Build history of the part. All positions in model axes, mm. A direction names the side the tool comes from. Round coordinates to 2 decimals unless told otherwise and drop trailing zeros. Loops run counter-clockwise (first coordinate to the right, second up) from the corner with the lowest first, then second, coordinate; pieces in that order, holes last. Notation, with made-up numbers: (82.5, 18.5) -> (87.5, 18.5) arc R20 cw to (87.5, 37.5) -> close; hole circle Ø4 at (27.25, -33.5). An arc over 180 degrees is marked (long way). Put each result on its own line as item: value. Start each with the question number.
```python
from build123d import *

# Parameters (mm, degrees)
SKETCH_1_W          = 480
SKETCH_1_H          = 178
EXTRUDE_1_DEPTH     = 2
SKETCH_2_R          = 3
CUT_EXTRUDE_1_DEPTH = 256.978514723
FILLET_1_R          = 5
SKETCH_3_W          = 430
SKETCH_3_H          = 128
CUT_EXTRUDE_2_DEPTH = 256.978514723
FILLET_2_R          = 30


with BuildPart() as part:
    # 草图1 → 凸台-拉伸1 (new body)
    with BuildSketch(Plane(origin=(0, 0, 0), x_dir=(0, 0, -1), z_dir=(1, 0, 0))):
        Rectangle(SKETCH_1_W, SKETCH_1_H)
    extrude(amount=EXTRUDE_1_DEPTH)

    # 草图2 → 切除-拉伸1 (cut, through all)
    with BuildSketch(Plane(origin=(2, 0, 0), x_dir=(0, 0, -1), z_dir=(1, 0, 0))):
        with Locations((-225, 74)):
            Circle(SKETCH_2_R)
        with Locations((225, 74)):
            Circle(SKETCH_2_R)
        with Locations((-225, -74)):
            Circle(SKETCH_2_R)
        with Locations((225, -74)):
            Circle(SKETCH_2_R)
    extrude(amount=-CUT_EXTRUDE_1_DEPTH, mode=Mode.SUBTRACT)

    # 圆角1
    fillet_1_edges = [part.edges().sort_by_distance(p)[0] for p in [
        (1, 89, 240),
        (1, 89, -240),
        (1, -89, -240),
        (1, -89, 240),
    ]]
    fillet(fillet_1_edges, radius=FILLET_1_R)

    # 草图3 → 切除-拉伸2 (cut, through all)
    with BuildSketch(Plane(origin=(2, 0, 0), x_dir=(0, 0, -1), z_dir=(1, 0, 0))):
        Rectangle(SKETCH_3_W, SKETCH_3_H)
    extrude(amount=-CUT_EXTRUDE_2_DEPTH, mode=Mode.SUBTRACT)

    # 圆角2
    fillet_2_edges = [part.edges().sort_by_distance(p)[0] for p in [
        (1, -64, 215),
        (1, 64, 215),
        (1, 64, -215),
        (1, -64, -215),
    ]]
    fillet(fillet_2_edges, radius=FILLET_2_R)


solid = part.part
```
Item 1: Cut at C-C on y = 52.5. Write the cut outline in (x, z), then the cut area to 3 significant figures.
Item 2: Cut at A-A on z = -110. Write the cut outline in (x, y).
Item 3: Cut at B-B on x = 1. Write the cut outline in (y, z).
Item 4: Pull direction Y, two halves, no side cores. Call faces 3 (the face through (0, 66, -17)), 4 (the face through (0.986, -55.445, -205.979)): +Y half, -Y half, draft (parallel to the pull), parting line (faces both ways), or undercut.
Item 5: Wall check: line 1 (Y direction, x = 1.6, z = 225); line 2 (Y direction, x = 1.55, z = 107.5); line 3 (Z direction, x = 1.3, y = -16). Give the ranges that are in metal, low to high. Write a range as from..to.
Item 6: 3-axis set-ups, long thin cutter, end or side, ignore diameter. For faces 1 (the face through (0.986, 55.445, 205.979)), 2 (the face through (2, 66, -17)): which of +Z, -Z, +X, -X, +Y, -Y reach the whole face in a straight line?
Ans:
1. outline: (0, -240) -> (2, -240) -> (2, -208.62) -> (0, -208.62) -> close; (0, 208.62) -> (2, 208.62) -> (2, 240) -> (0, 240) -> close
1. area: 126 mm2
2. outline: (0, -89) -> (2, -89) -> (2, -64) -> (0, -64) -> close; (0, 64) -> (2, 64) -> (2, 89) -> (0, 89) -> close
3. outline: (-89, -235) arc R5 ccw to (-84, -240) -> (84, -240) arc R5 ccw to (89, -235) -> (89, 235) arc R5 ccw to (84, 240) -> (-84, 240) arc R5 ccw to (-89, 235) -> close; hole circle Ø6 at (-74, -225); hole circle Ø6 at (-74, 225); hole (-64, -185) arc R30 ccw to (-34, -215) -> (34, -215) arc R30 ccw to (64, -185) -> (64, 185) arc R30 ccw to (34, 215) -> (-34, 215) arc R30 ccw to (-64, 185) -> close; hole circle Ø6 at (74, -225); hole circle Ø6 at (74, 225)
4. face 3: draft
4. face 4: undercut
5. line 1: y = -89..-77, -71..71, 77..89
5. line 2: y = -89..-64, 64..89
5. line 3: z = -240..-215, 215..240
6. face 1: +X, -X
6. face 2: +Z, -Z, +X, +Y, -Y
